Input: part model. Units: mm. Frame: model coordinates. Round coordinates to 2 decimals unless told otherwise and drop trailing zeros. Loops run counter-clockwise (first coordinate to the right, second up) from the corner with the lowest first, then second, coordinate; pieces in that order, holes last.
1) First-contact query: pin 1 (4 mm diameter, centred on x = -20, z = -25, fed in from +Y); pin 2 (6 mm diameter, centred on y = 9, z = -344, fed in from +X); pin 3 (3 mm diameter, centred on x = -1, z = -475, fed in from -Y); pin 4 (0.8 mm diameter, centred on x = -11.5, z = -419.5, fed in from +Y). Flat tips, straight axial feed; report the tip coordinate or a pass-through.
2) Ray query, line 1 along X through (y, z) = (5, -25); line 2 along Z through (x, y) = (0, 5); line 3 along Z through (x, y) = (-20, 3.75). Return the intervals inside material, ascending.
3) Section A-A, the plane z = -142.5. Return loops of the section in (x, y), and give its area (3 significant figures).
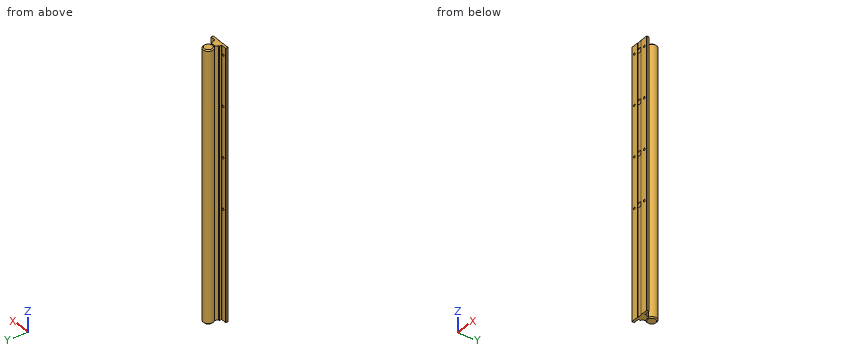
from build123d import *

# Parameters (mm, degrees)
SKETCH6_R                      = 15
BOSS_EXTRUDE2_DEPTH            = 800
CHAMFER1_SIZE                  = 3
BOSS_EXTRUDE1_DEPTH            = 800
SKETCH4_W                      = 3.3
SKETCH4_H                      = 7
CURVE_PATTERN1_COUNT           = 4
CURVE_PATTERN1_PITCH           = 150
CURVE_PATTERN1_COPY_1_SKETCH_W = 3.3
CURVE_PATTERN1_COPY_1_SKETCH_H = 7
CURVE_PATTERN1_COPY_2_SKETCH_W = 3.3
CURVE_PATTERN1_COPY_2_SKETCH_H = 7
CURVE_PATTERN1_COPY_3_SKETCH_W = 3.3
CURVE_PATTERN1_COPY_3_SKETCH_H = 7


with BuildPart() as part:
    # Sketch6 → Boss-Extrude2 (new body)
    with BuildSketch(Plane.XY):
        with Locations((0, 37)):
            Circle(SKETCH6_R)
    extrude(amount=-BOSS_EXTRUDE2_DEPTH)

    # Chamfer1
    chamfer1_edges = [part.edges().sort_by_distance(p)[0] for p in [
        (-15, 37, 0),
        (-15, 37, -800),
    ]]
    chamfer(chamfer1_edges, length=CHAMFER1_SIZE)

    # Sketch3 → Boss-Extrude1 (add)
    with BuildSketch(Plane.XY):
        with BuildLine():
            Line((-10.499533732, 14.404167217), (-6.30880391, 23.391216321))
            ThreePointArc((-6.30880391, 23.391216321), (0, 22), (6.30880391, 23.391216321))
            Line((6.30880391, 23.391216321), (10.499533732, 14.404167217))
            ThreePointArc((10.499533732, 14.404167217), (10.757839457, 14.109625988), (11.133949183, 14))
            Line((11.133949183, 14), (12.66, 14))
            ThreePointArc((12.66, 14), (13.154974747, 13.794974747), (13.36, 13.3))
            Line((13.36, 13.3), (13.36, 7.7))
            ThreePointArc((13.36, 7.7), (13.565025253, 7.205025253), (14.06, 7))
            Line((14.06, 7), (29.3, 7))
            ThreePointArc((29.3, 7), (29.794974747, 6.794974747), (30, 6.3))
            Line((30, 6.3), (30, 0.7))
            ThreePointArc((30, 0.7), (29.794974747, 0.205025253), (29.3, 0))
            Line((29.3, 0), (7, 0))
            Line((7, 0), (7, 0.7))
            Line((7, 0.7), (-7, 0.7))
            Line((-7, 0.7), (-7, 0))
            Line((-7, 0), (-29.3, 0))
            ThreePointArc((-29.3, 0), (-29.794974747, 0.205025253), (-30, 0.7))
            Line((-30, 0.7), (-30, 6.3))
            ThreePointArc((-30, 6.3), (-29.794974747, 6.794974747), (-29.3, 7))
            Line((-29.3, 7), (-14.06, 7))
            ThreePointArc((-14.06, 7), (-13.565025253, 7.205025253), (-13.36, 7.7))
            Line((-13.36, 7.7), (-13.36, 13.3))
            ThreePointArc((-13.36, 13.3), (-13.154974747, 13.794974747), (-12.66, 14))
            Line((-12.66, 14), (-11.133949183, 14))
            ThreePointArc((-11.133949183, 14), (-10.757839457, 14.109625988), (-10.499533732, 14.404167217))
        make_face()
    extrude(amount=-BOSS_EXTRUDE1_DEPTH)

    # Sketch4 → Cut-Revolve1 (revolve, cut)
    with BuildSketch(Plane.XY.offset(-25), mode=Mode.PRIVATE) as cut_revolve1_sk:
        with Locations((-21.65, 3.5)):
            Rectangle(SKETCH4_W, SKETCH4_H)
    cut_revolve1 = revolve(cut_revolve1_sk.sketch.rotate(Axis((-20, 7, -25), (0, -1, 0)), 270), axis=Axis((-20, 7, -25), (0, -1, 0)), mode=Mode.SUBTRACT)

    # Mirror1: Cut-Revolve1 across plane
    add(cut_revolve1.mirror(Plane(origin=(0, 0, 0), x_dir=(0, 0, 1), z_dir=(1, 0, 0))), mode=Mode.SUBTRACT)

    # Sketch5 → Cut-Revolve2 (revolve, cut)
    with BuildSketch(Plane.XY.offset(-25)):
        Polygon((-7, 0.7), (-7, 9.1), (-2.8, 9.1), (-2.8, 34.475681392), (0, 34.475681392), (0, 0.7), align=None)
    cut_revolve2 = revolve(axis=Axis((0, 34.475681392, -25), (0, -1, 0)), mode=Mode.SUBTRACT)

    # Curve Pattern1: Cut-Revolve1, Cut-Revolve2 ×4
    with Locations(*[(0, 0, -i * CURVE_PATTERN1_PITCH) for i in range(1, CURVE_PATTERN1_COUNT)]):
        add(cut_revolve1, mode=Mode.SUBTRACT)
        add(cut_revolve2, mode=Mode.SUBTRACT)

    # Curve Pattern1 copy 1 sketch → Curve Pattern1 copy 1 (revolve, cut)
    with BuildSketch(Plane(origin=(0, 0, -175), x_dir=(-1, 0, 0), z_dir=(0, 0, 1))):
        with Locations((-21.65, -3.5)):
            Rectangle(CURVE_PATTERN1_COPY_1_SKETCH_W, CURVE_PATTERN1_COPY_1_SKETCH_H)
    revolve(axis=Axis((20, 7, -175), (0, 1, 0)), mode=Mode.SUBTRACT)

    # Curve Pattern1 copy 2 sketch → Curve Pattern1 copy 2 (revolve, cut)
    with BuildSketch(Plane(origin=(0, 0, -325), x_dir=(-1, 0, 0), z_dir=(0, 0, 1))):
        with Locations((-21.65, -3.5)):
            Rectangle(CURVE_PATTERN1_COPY_2_SKETCH_W, CURVE_PATTERN1_COPY_2_SKETCH_H)
    revolve(axis=Axis((20, 7, -325), (0, 1, 0)), mode=Mode.SUBTRACT)

    # Curve Pattern1 copy 3 sketch → Curve Pattern1 copy 3 (revolve, cut)
    with BuildSketch(Plane(origin=(0, 0, -475), x_dir=(-1, 0, 0), z_dir=(0, 0, 1))):
        with Locations((-21.65, -3.5)):
            Rectangle(CURVE_PATTERN1_COPY_3_SKETCH_W, CURVE_PATTERN1_COPY_3_SKETCH_H)
    revolve(axis=Axis((20, 7, -475), (0, 1, 0)), mode=Mode.SUBTRACT)


solid = part.part
Final values:
1. pin 1: passes through
1. pin 2: stops at x = 30
1. pin 3: stops at y = 34.48
1. pin 4: stops at y = 47.09
2. line 1: x = -30 to -23.3, -16.7 to -7, 7 to 16.7, 23.3 to 30
2. line 2: z = -800 to -482, -468 to -332, -318 to -182, -168 to -32, -18 to 0
2. line 3: z = -800 to -478.3, -471.7 to -328.3, -321.7 to -178.3, -171.7 to -28.3, -21.7 to 0
3. outline: (-30, 0.7) arc R0.7 ccw to (-29.3, 0) - (-7, 0) - (-7, 0.7) - (7, 0.7) - (7, 0) - (29.3, 0) arc R0.7 ccw to (30, 0.7) - (30, 6.3) arc R0.7 ccw to (29.3, 7) - (14.06, 7) arc R0.7 cw to (13.36, 7.7) - (13.36, 13.3) arc R0.7 ccw to (12.66, 14) - (11.13, 14) arc R0.7 cw to (10.5, 14.4) - (6.31, 23.39) arc R15 ccw (long way) to (-6.31, 23.39) - (-10.5, 14.4) arc R0.7 cw to (-11.13, 14) - (-12.66, 14) arc R0.7 ccw to (-13.36, 13.3) - (-13.36, 7.7) arc R0.7 cw to (-14.06, 7) - (-29.3, 7) arc R0.7 ccw to (-30, 6.3) - close
3. area: 1,450 mm2
